Geometry check sheet. Reference: the model listing, model coordinates, mm. Round coordinates to 2 decimals unless told otherwise and drop trailing zeros. Loops run counter-clockwise (first coordinate to the right, second up) from the corner with the lowest first, then second, coordinate; pieces in that order, holes last. Notation, with made-up numbers: (-36.5, 67) - (-25.5, 67) arc R16 ccw to (-25.5, 82) - close; hole circle Ø11 at (4.25, 55). An arc over 180 degrees is marked (long way). Write item = value, one per line.
```python
from build123d import *

# Parameters (mm, degrees)
SKETCH_1_W          = 160
SKETCH_1_H          = 170
EXTRUDE_1_DEPTH     = 24
HOLE_WIZARD_M16_1_D = 14


with BuildPart() as part:
    # 草图1 → 凸台-拉伸1 (new body)
    with BuildSketch(Plane(origin=(0, 0, 0), x_dir=(1, 0, 0), z_dir=(0, 1, 0))):
        Rectangle(SKETCH_1_W, SKETCH_1_H)
    extrude(amount=EXTRUDE_1_DEPTH)

    # M16 螺纹孔1 (through all)
    with Locations(Plane(origin=(0, 24, 0), x_dir=(1, 0, 0), z_dir=(0, 1, 0))):
        with Locations((-55, -60), (-55, 60), (55, 60), (55, -60), (55, 0), (-55, 0)):
            Hole(HOLE_WIZARD_M16_1_D / 2)


solid = part.part
```
(1) Gauge pin test, flat end, axial feed: pin 1 (10 mm diameter, centred on x = 9, z = 30.5, fed in from -Y). Record the tip position at first contact, or that the pin passes through.
Answers follow:
pin_1 = 0
(2) Section check B-B (z = 60). Enter the section's corners in (x, y), then the cut area to 3 significant figures.
Answers follow:
outline = (-80, 0) - (-62, 0) - (-62, 24) - (-80, 24) - close; (-48, 0) - (48, 0) - (48, 24) - (-48, 24) - close; (62, 0) - (80, 0) - (80, 24) - (62, 24) - close
area = 3,170 mm²
(3) Section check C-C (y = 9). Enter the section's corners in (x, z), then the cut area to 3 significant figures.
Answers follow:
outline = (-80, -85) - (80, -85) - (80, 85) - (-80, 85) - close; hole circle Ø14 at (-55, -60); hole circle Ø14 at (-55, 0); hole circle Ø14 at (-55, 60); hole circle Ø14 at (55, -60); hole circle Ø14 at (55, 0); hole circle Ø14 at (55, 60)
area = 26,300 mm²
(4) Mould release check, pull along Z, two halves, no side actions. Record for faces 1 (the flat face through (-80, 12, 1)), 2 (the cylindrical face through (-54.09, 11.83, -66.94)), 3 (the flat face through (-1, 12, 85)): pulls with the +Z half, pulls with the -Z half, needs draft (parallel to the pull), parting line crosses it, or undercut.
Answers follow:
face_1 = needs draft
face_2 = undercut
face_3 = pulls with the +Z half
(5) Section check A-A (x = 55). Enter the section's corners in (y, z), then the cut area to 3 significant figures.
Answers follow:
outline = (0, -85) - (24, -85) - (24, -67) - (0, -67) - close; (0, -53) - (24, -53) - (24, -7) - (0, -7) - close; (0, 7) - (24, 7) - (24, 53) - (0, 53) - close; (0, 67) - (24, 67) - (24, 85) - (0, 85) - close
area = 3,070 mm²
(6) Scan lines: L1, parallel to X at y = 8.25, z = 60; L2, parallel to Z at x = -55, y = 9; L3, parallel to X at y = 8.75, z = -64. Record each from-to range of solid material in increasing order. Write a range as [from, to].
Answers follow:
L1 = [-80, -62], [-48, 48], [62, 80]
L2 = [-85, -67], [-53, -7], [7, 53], [67, 85]
L3 = [-80, -60.74], [-49.26, 49.26], [60.74, 80]
